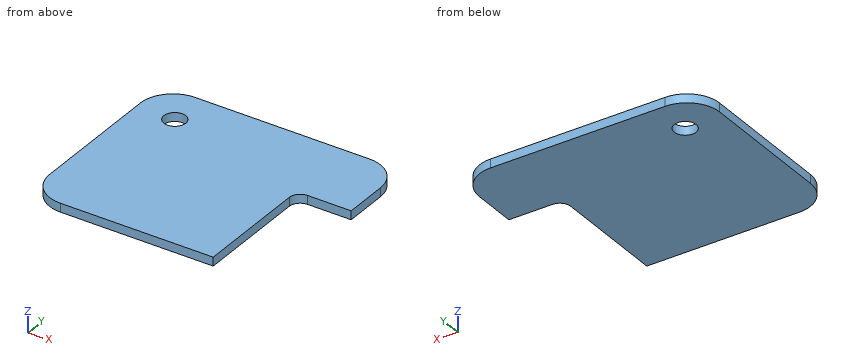
from build123d import *

# Parameters (mm, degrees)
SKETCH_1_R      = 10
EXTRUDE_1_DEPTH = 8


with BuildPart() as part:
    # 草图1 → 凸台-拉伸1 (new body)
    with BuildSketch(Plane.XY):
        with BuildLine():
            Line((0, 30), (0, 154))
            ThreePointArc((0, 154), (8.786796564, 175.213203436), (30, 184))
            Line((30, 184), (190, 184))
            ThreePointArc((190, 184), (211.213203436, 175.213203436), (220, 154))
            Line((220, 154), (220, 114))
            Line((220, 114), (180, 114))
            ThreePointArc((180, 114), (172.928932188, 111.071067812), (170, 104))
            Line((170, 104), (170, 0))
            Line((170, 0), (30, 0))
            ThreePointArc((30, 0), (8.786796564, 8.786796564), (0, 30))
        make_face()
        with Locations((35, 149)):
            Circle(SKETCH_1_R, mode=Mode.SUBTRACT)
    extrude(amount=EXTRUDE_1_DEPTH)


solid = part.part
Model file for the job. Use its own axes, mm. Round coordinates to 2 decimals unless told otherwise and drop trailing zeros. Order: outer loops, then holes, each group sorted by start corner. A loop starts at its lowest first (then second) coordinate and runs counter-clockwise, first axis right, second up.
(1) Band-saw the part on C-C (y = 149). List the corners of the cut face in (x, z), then the cut area to 3 significant figures.
(2) Drill centre lines: line 1 (Y direction, x = 35, z = 6); line 2 (X direction, y = 97, z = 6.25); line 3 (X direction, y = 10, z = 7.75). Where is each one in solid material? Low to high.
(3) Band-saw the part on A-A (x = 35). List the corners of the cut face in (y, z).
(4) Pin check, flat tips, straight feed: pin 1 (2.5 mm diameter, centred on x = 203.5, z = 4.5, fed in from -Y); pin 2 (2.5 mm diameter, centred on y = 39.5, z = 4, fed in from +X); pin 3 (12 mm diameter, centred on x = 35, y = 149, fed in from -Z). Stop position of each tip, or through.
(5) Band-saw the part on B-B (z = 2). List the corners of the cut face in (x, y).
(6) Band-saw the part on D-D (y = 45). List the corners of the cut face in (x, z), then the cut area to 3 significant figures.
Verdict:
1. outline: (0, 0) - (25, 0) - (25, 8) - (0, 8) - close; (45, 0) - (220, 0) - (220, 8) - (45, 8) - close
1. area: 1,600 mm2
2. line 1: y = 0 to 139, 159 to 184
2. line 2: x = 0 to 170
2. line 3: x = 7.64 to 170
3. outline: (0, 0) - (139, 0) - (139, 8) - (0, 8) - close; (159, 0) - (184, 0) - (184, 8) - (159, 8) - close
4. pin 1: stops at y = 114
4. pin 2: stops at x = 170
4. pin 3: passes through
5. outline: (0, 30) arc R30 ccw to (30, 0) - (170, 0) - (170, 104) arc R10 cw to (180, 114) - (220, 114) - (220, 154) arc R30 ccw to (190, 184) - (30, 184) arc R30 ccw to (0, 154) - close; hole circle Ø20 at (35, 149)
6. outline: (0, 0) - (170, 0) - (170, 8) - (0, 8) - close
6. area: 1,360 mm2
